from build123d import *

# Parameters (mm, degrees)
SKETCH1_R           = 8.5
BOSS_EXTRUDE1_DEPTH = 4
SKETCH2_R           = 9
BOSS_EXTRUDE2_DEPTH = 2.8
FILLET1_R           = 0.3
SKETCH3_R           = 1.5
CUT_EXTRUDE1_DEPTH  = 5


with BuildPart() as part:
    # Sketch1 → Boss-Extrude1 (new body)
    with BuildSketch(Plane.XY):
        Circle(SKETCH1_R)
    extrude(amount=BOSS_EXTRUDE1_DEPTH)

    # Sketch2 → Boss-Extrude2 (add)
    with BuildSketch(Plane.XY.offset(4)):
        Circle(SKETCH2_R)
    extrude(amount=BOSS_EXTRUDE2_DEPTH)

    # Fillet1
    fillet1_edges = [part.edges().sort_by_distance(p)[0] for p in [
        (-9, 0, 4),
        (-9, 0, 6.8),
    ]]
    fillet(fillet1_edges, radius=FILLET1_R)

    # Sketch3 → Cut-Extrude1 (cut)
    with BuildSketch(Plane(origin=(0, 0, 0), x_dir=(-1, 0, 0), z_dir=(0, 0, -1))):
        Circle(SKETCH3_R)
    extrude(amount=-CUT_EXTRUDE1_DEPTH, mode=Mode.SUBTRACT)


solid = part.part
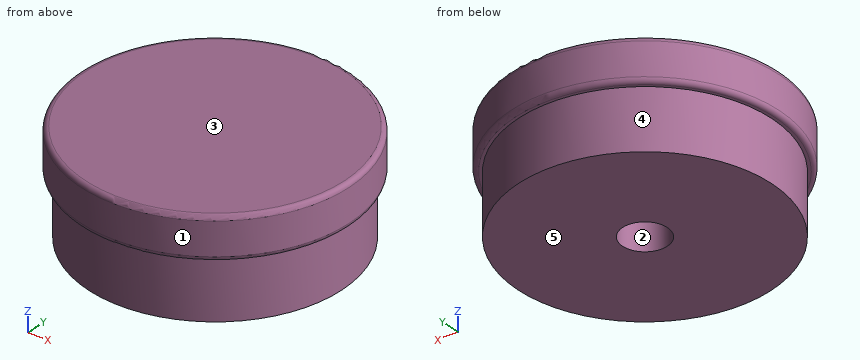
Can you work these out from the model? Positions are in its coordinate system, mm. Face numbers are marked on the shaded views. A direction names the side the tool comes from. Coordinates: 2 decimals unless noted, no trailing zeros. Loops run counter-clockwise (first coordinate to the right, second up) from the corner with the lowest first, then second, coordinate; pieces in that order, holes last. Notation, with made-up numbers: M 14,72 L 54,72 A29 ccw 54,101 Z; hole C 10,4 d4. An arc over 180 degrees is marked long. Return JSON: item names as keys, results as strings. Group by question number.
Item 1: I'm going to push flat-ended pins straight in: pin 1 Ø2 at (y, z) = (-5, 5) entering from -X; pin 2 Ø2 at (y, z) = (2, 1.5) entering from +X; pin 3 Ø1 at (x, z) = (-5.5, 6) entering from -Y. Where does each tip first touch, or does it pass through?
Item 2: Imagine slicing it at C-C (z = 1.25). Please give me the cut outline in (x, y), and give its area (3 significant figures).
Item 3: If I drill on L1, parallel to Y at x = 0, z = 1.75; L2, parallel to Z at x = -7, y = 5.25; L3, parallel to X at y = -7.5, z = 3.5, over which ranges is the centre line in solid material (lowest first)? Write a range as from..to.
Item 4: Imagine slicing it at D-D (z = 6). Please give me the cut outline in (x, y).
Item 5: Thinking about a two-plate mould opening in X: for the marked faces 1, 2 and 3, which applies, released by +X, released by -X, zero draft, split by the parting line, or undercut?
Item 6: On a 3-axis mill with a long thin cutter (end or side, diameter ignored), from which of +Z, -Z, +X, -X, +Y, -Y can I reach the whole of each face in a straight line? I mean the marked faces 4 and 5. Say none if no direction works.
Item 7: Imagine slicing it at A-A (x = 0). Please give me the cut outline in (y, z), and give its area (3 significant figures).
Verdict:
{
 "1": {"pin 1": "stops at x = -8.06", "pin 2": "stops at x = 8.44", "pin 3": "stops at y = -7.48"},
 "2": {"outline": "C 0,0 d17; hole C 0,0 d3", "area": "220 mm^2"},
 "3": {"L1": "y = -8.5..-1.5, 1.5..8.5", "L2": "z = 4..6.8", "L3": "x = -4..4"},
 "4": {"outline": "C 0,0 d18"},
 "5": {"face 1": "split by the parting line", "face 2": "undercut", "face 3": "zero draft"},
 "6": {"face 4": "-Z", "face 5": "-Z, +X, -X, +Y, -Y"},
 "7": {"outline": "M -9,4.3 A0.3 ccw -8.7,4 L -8.5,4 L -8.5,0 L -1.5,0 L -1.5,5 L 1.5,5 L 1.5,0 L 8.5,0 L 8.5,4 L 8.7,4 A0.3 ccw 9,4.3 L 9,6.5 A0.3 ccw 8.7,6.8 L -8.7,6.8 A0.3 ccw -9,6.5 Z", "area": "103 mm^2"}
}
